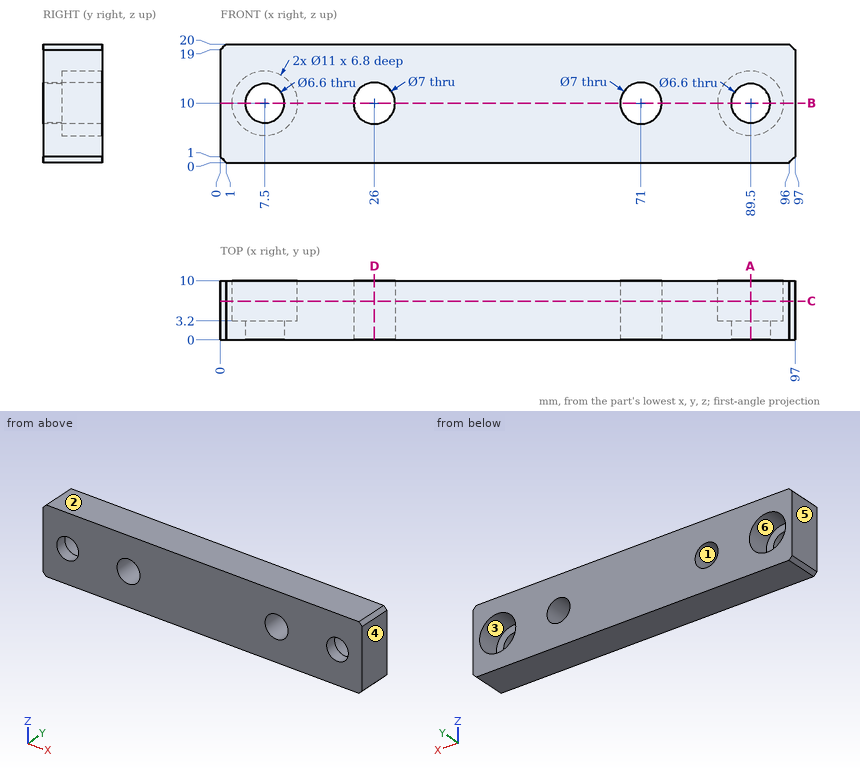
Source: three-view drawing plus pictorial views. Frame: mm from the lowest corner of the part. A direction names the side the tool comes from. Round coordinates to 2 decimals unless told otherwise and drop trailing zeros. Loops run counter-clockwise (first coordinate to the right, second up) from the corner with the lowest first, then second, coordinate; pieces in that order, holes last.
Q1. Section D-D on x = 26. Return loops of the section in (y, z), plus the area to 3 significant figures.
Q2. Section B-B on z = 10. Return loops of the section in (x, y).
Q3. Section A-A on x = 89.5. Return loops of the section in (y, z), plus the area to 3 significant figures.
Q4. Pull-direction query (X, two-part tool) for the marked faces 1, 2, 3 and 4; classes: released by +X, released by -X, zero draft, split by the parting line, or undercut.
Q5. Section C-C on y = 6.5. Return loops of the section in (x, z), plus the area to 3 significant figures.
Q6. Material intervals for L1, parallel to X at y = 1.5, z = 11; L2, parallel to Z at x = 26, y = 4.5; L3, parallel to Z at x = 89.5, y = 7.75, sorted ascending.
Q7. Pin query (flat end, axial travel): P1, Ø10.5, axis at x = 7.5, z = 10, coming from the +Y side. Return the tip coordinate at first contact, or that it passes through.
Q8. Access query for the marked faces 5 and 6. Directions: +Z, -Z, +X, -X, +Y, -Y. A direction counts if a zero-diameter tool reaches every point of the face in a straight line with its end or side. Return the directions, or none.
Evaluation:
1. outline: (0, 0) - (10, 0) - (10, 6.5) - (0, 6.5) - close; (0, 13.5) - (10, 13.5) - (10, 20) - (0, 20) - close
1. area: 130 mm2
2. outline: (0, 0) - (4.2, 0) - (4.2, 3.2) - (2, 3.2) - (2, 10) - (0, 10) - close; (10.8, 0) - (22.5, 0) - (22.5, 10) - (13, 10) - (13, 3.2) - (10.8, 3.2) - close; (29.5, 0) - (67.5, 0) - (67.5, 10) - (29.5, 10) - close; (74.5, 0) - (86.2, 0) - (86.2, 3.2) - (84, 3.2) - (84, 10) - (74.5, 10) - close; (92.8, 0) - (97, 0) - (97, 10) - (95, 10) - (95, 3.2) - (92.8, 3.2) - close
3. outline: (0, 0) - (10, 0) - (10, 4.5) - (3.2, 4.5) - (3.2, 6.7) - (0, 6.7) - close; (0, 13.3) - (3.2, 13.3) - (3.2, 15.5) - (10, 15.5) - (10, 20) - (0, 20) - close
3. area: 104 mm2
4. face 1: undercut
4. face 2: zero draft
4. face 3: undercut
4. face 4: released by +X
5. outline: (0, 1) - (1, 0) - (96, 0) - (97, 1) - (97, 19) - (96, 20) - (1, 20) - (0, 19) - close; hole circle Ø11 at (7.5, 10); hole circle Ø7 at (26, 10); hole circle Ø7 at (71, 10); hole circle Ø11 at (89.5, 10)
5. area: 1,670 mm2
6. L1: x = 0 to 4.36, 10.64 to 22.65, 29.35 to 67.65, 74.35 to 86.36, 92.64 to 97
6. L2: z = 0 to 6.5, 13.5 to 20
6. L3: z = 0 to 4.5, 15.5 to 20
7. P1: stops at y = 3.2
8. face 5: +Z, -Z, -X, +Y, -Y
8. face 6: +Y
